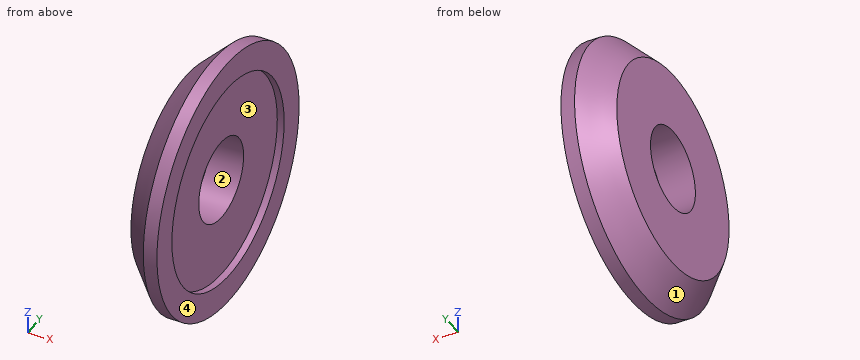
from build123d import *


with BuildPart() as part:
    # Sketch1 → Revolve2 (revolve)
    with BuildSketch(Plane.XY, mode=Mode.PRIVATE) as revolve2_sk:
        Polygon((-3, 15), (-3, 6), (2, 6), (2, 15), (3, 15), (3, 19), (1, 19), align=None)
    revolve(revolve2_sk.sketch.rotate(Axis((-11.259866943, 0, 0), (1, 0, 0)), 90), axis=Axis((-11.259866943, 0, 0), (1, 0, 0)))


solid = part.part
Build history of the part. All positions in model axes, mm. Face numbers are marked on the shaded views. Round coordinates to 2 decimals unless told otherwise and drop trailing zeros. Write each loop counter-clockwise with the first axis right and the second up, starting at its lowest first coordinate (ties: lowest second). Pieces come first, ordered by that corner, then holes. Notation, with made-up numbers: (37.5, 34.5) -> (72.5, 34.5) arc R10 cw to (72.5, 47.5) -> close; hole circle Ø7 at (18, -5). An arc over 180 degrees is marked (long way). Use one line per item in the form item = value.
Q1. Band-saw the part on D-D, the plane x = -2.25. Write the cut outline in (y, z), then the cut area to 3 significant figures.
Conclusion:
outline = circle Ø31.5 at (0, 0); hole circle Ø12 at (0, 0)
area = 666 mm²
Q2. Band-saw the part on A-A, the plane y = 0. Write the cut outline in (x, z).
Conclusion:
outline = (-3, -15) -> (1, -19) -> (3, -19) -> (3, -15) -> (2, -15) -> (2, -6) -> (-3, -6) -> close; (-3, 6) -> (2, 6) -> (2, 15) -> (3, 15) -> (3, 19) -> (1, 19) -> (-3, 15) -> close
Q3. Drill centre lines: L1, parallel to Y at x = 2.55, z = 0; L2, parallel to Z at x = 1.5, y = 2.5; L3, parallel to Z at x = -1.25, y = -2. Where is each one in solid material? Low to high.
Conclusion:
L1 = -19 to -15, 15 to 19
L2 = -18.83 to -5.45, 5.45 to 18.83
L3 = -16.63 to -5.66, 5.66 to 16.63
Q4. Two-plate mould, pull along Z, no slides. Class the marked faces 1, 2, 3 and 4: released by +Z, released by -Z, zero draft, split by the parting line, or undercut.
Conclusion:
face_1 = split by the parting line
face_2 = undercut
face_3 = undercut
face_4 = zero draft
Q5. Drop flat-ended pins along their axis: P1, Ø1.5, axis at x = 2, z = -13, coming from the +Y side; P2, Ø3, axis at x = 0.5, z = -6, coming from the +Y side; P3, Ø4, axis at y = 3.5, z = 7, coming from the +X side. Give the stop position or say it passes through.
Conclusion:
P1 = 14.52
P2 = 18.44
P3 = 2
Q6. Band-saw the part on C-C, the plane x = 1.5. Write the cut outline in (y, z), then the cut area to 3 significant figures.
Conclusion:
outline = circle Ø38 at (0, 0); hole circle Ø12 at (0, 0)
area = 1,020 mm²
